The listing builds one solid part. Answer for the finished solid, in the listing's coordinates (mm). A direction names the side the tool comes from. Coordinates: 2 decimals unless noted, no trailing zeros. Loops run counter-clockwise (first coordinate to the right, second up) from the corner with the lowest first, then second, coordinate; pieces in that order, holes last. Notation, with made-up numbers: (18, 22) - (32, 22) arc R11 cw to (32, 41) - close; hole circle Ø10 at (35.5, -21). An arc over 180 degrees is marked (long way). One line per question, with ' | ' between items.
from build123d import *

# Parameters (mm, degrees)
SKETCH_1_W          = 2266
SKETCH_1_H          = 327.5
EXTRUDE_1_DEPTH     = 40
SKETCH_2_W          = 430
SKETCH_2_H          = 350
EXTRUDE_2_DEPTH     = 40
CUT_EXTRUDE_1_DEPTH = 1245.67990363
FILLET_1_R          = 30


with BuildPart() as part:
    # 草图1 → 凸台-拉伸1 (new body)
    with BuildSketch(Plane(origin=(0, 0, 0), x_dir=(1, 0, 0), z_dir=(0, 1, 0))):
        Rectangle(SKETCH_1_W, SKETCH_1_H)
    extrude(amount=EXTRUDE_1_DEPTH)

    # 草图2 → 凸台-拉伸2 (add)
    with BuildSketch(Plane(origin=(0, 40, 0), x_dir=(1, 0, 0), z_dir=(0, 1, 0))):
        with Locations((-648, -338.75)):
            Rectangle(SKETCH_2_W, SKETCH_2_H)
    extrude(amount=-EXTRUDE_2_DEPTH)

    # 草图3 → 切除-拉伸1 (cut, through all)
    with BuildSketch(Plane(origin=(0, 40, 0), x_dir=(1, 0, 0), z_dir=(0, 1, 0))):
        with BuildLine():
            Line((-503, -187.75), (-503, -237.75))
            ThreePointArc((-503, -237.75), (-514, -248.75), (-525, -237.75))
            Line((-525, -237.75), (-525, -187.75))
            ThreePointArc((-525, -187.75), (-514, -176.75), (-503, -187.75))
        make_face()
        with BuildLine():
            Line((-787, -187.75), (-787, -237.75))
            ThreePointArc((-787, -237.75), (-798, -248.75), (-809, -237.75))
            Line((-809, -237.75), (-809, -187.75))
            ThreePointArc((-809, -187.75), (-798, -176.75), (-787, -187.75))
        make_face()
        with BuildLine():
            Line((-787, -439.75), (-787, -489.75))
            ThreePointArc((-787, -489.75), (-798, -500.75), (-809, -489.75))
            Line((-809, -489.75), (-809, -439.75))
            ThreePointArc((-809, -439.75), (-798, -428.75), (-787, -439.75))
        make_face()
        with BuildLine():
            Line((-503, -439.75), (-503, -489.75))
            ThreePointArc((-503, -489.75), (-514, -500.75), (-525, -489.75))
            Line((-525, -489.75), (-525, -439.75))
            ThreePointArc((-525, -439.75), (-514, -428.75), (-503, -439.75))
        make_face()
    extrude(amount=-CUT_EXTRUDE_1_DEPTH, mode=Mode.SUBTRACT)

    # 圆角1
    fillet_1_edges = [part.edges().sort_by_distance(p)[0] for p in [
        (-433, 20, 163.75),
        (-863, 20, 163.75),
    ]]
    fillet(fillet_1_edges, radius=FILLET_1_R)


solid = part.part
Item 1: Which of the six approach directions +Z, -Z, +X, -X, +Y, -Y give full straight-line access (tool end or side, diameter ignored) to faces 4 (the face through (-809, 20, 213)), 5 (the face through (-1015, 20, 163.75)), 6 (the face through (354, 20, 163.75))?
Taken from the geometry:
face 4: +Y, -Y | face 5: +Z, -X, +Y, -Y | face 6: +Z, +X, +Y, -Y
Item 2: Each of these flat-tipped pins is pushed along its axis until it touches: pin 1 Ø1 at (x, y) = (-278.5, 4.5) entering from +Z; pin 2 Ø20 at (y, z) = (18, 216.5) entering from -X; pin 3 Ø12 at (y, z) = (24.5, 203.5) entering from +X. Where does it stop, or does it pass through?
Taken from the geometry:
pin 1: stops at z = 163.75 | pin 2: stops at x = -863 | pin 3: stops at x = -433
Item 3: Find section A-A, the plane y = 23. Write down the section's boundary in (x, z), plus the area to 3 significant figures.
Taken from the geometry:
outline: (-1133, -163.75) - (1133, -163.75) - (1133, 163.75) - (-403, 163.75) arc R30 cw to (-433, 193.75) - (-433, 513.75) - (-863, 513.75) - (-863, 193.75) arc R30 cw to (-893, 163.75) - (-1133, 163.75) - close; hole (-809, 187.75) arc R11 ccw to (-787, 187.75) - (-787, 237.75) arc R11 ccw to (-809, 237.75) - close; hole (-809, 439.75) arc R11 ccw to (-787, 439.75) - (-787, 489.75) arc R11 ccw to (-809, 489.75) - close; hole (-525, 187.75) arc R11 ccw to (-503, 187.75) - (-503, 237.75) arc R11 ccw to (-525, 237.75) - close; hole (-525, 439.75) arc R11 ccw to (-503, 439.75) - (-503, 489.75) arc R11 ccw to (-525, 489.75) - close | area: 887,000 mm2
Item 4: Find section B-B, the plane x = 465.5. Write down the section's boundary in (y, z).
Taken from the geometry:
outline: (0, -163.75) - (40, -163.75) - (40, 163.75) - (0, 163.75) - close
Item 5: The mould has two halves that part along X. Classify faces 1 (the face through (-1133, 20, 2)), 2 (the face through (-433, 20, 356)), 3 (the face through (-787, 20, 464)): pulls with the +X half, pulls with the -X half, needs draft (parallel to the pull), parting line crosses it, or undercut.
Taken from the geometry:
face 1: pulls with the -X half | face 2: pulls with the +X half | face 3: undercut
Item 6: Find the intervals of material crossed by line 1 (X direction, y = 20, z = 439); line 2 (X direction, y = 27, z = 374); line 3 (Z direction, x = -267, y = 7), in increasing order. Write a range as [from, to].
Taken from the geometry:
line 1: x = [-863, -808.97], [-787.03, -524.97], [-503.03, -433] | line 2: x = [-863, -433] | line 3: z = [-163.75, 163.75]
